Work out the finished part from the listing and answer in its coordinate system (mm). Give positions to 0.01 mm unless a question says otherwise; leave off trailing zeros. Order: outer loops, then holes, each group sorted by start corner. A loop starts at its lowest first (then second) coordinate and runs counter-clockwise, first axis right, second up. Notation, with made-up numbers: (80, 50.25) -> (90, 50.25) arc R24 cw to (90, 87.25) -> close; hole circle Ø6 at (-23, 40). An arc over 180 degrees is marked (long way). Answer as CSV lines item,"result". Start each with the question number.
1. A cutting plane is placed at A-A (y = 316). Give the vertices of the cut face in (x, z), then the cut area to 3 significant figures.
2. A flat-ended cylindrical pin translates along its axis: pin 1 (6 mm diameter, centred on x = 29, y = 284.5, fed in from +Z). Find the tip coordinate at first contact, or state that the pin passes through.
3. A cutting plane is placed at B-B (x = -35). Give the vertices of the cut face in (y, z) (3 decimals).
4. Find the intervals of material crossed by L1, parallel to Z at x = -33.5, y = 298; L2, parallel to Z at x = -36, y = 370; L3, parallel to X at y = 58.5, z = -35 (3 decimals), in increasing order.
5. A cutting plane is placed at C-C (z = 34.5). Give the vertices of the cut face in (x, y).
from build123d import *

# Parameters (mm, degrees)
BOSS_EXTRUDE1_DEPTH = 420


with BuildPart() as part:
    # Sketch1 → Boss-Extrude1 (new body)
    with BuildSketch(Plane.XZ):
        with BuildLine():
            Line((40, -26.666666667), (40, 26.666666667))
            ThreePointArc((40, 26.666666667), (36.094757082, 36.094757082), (26.666666667, 40))
            Line((26.666666667, 40), (-26.666666667, 40))
            ThreePointArc((-26.666666667, 40), (-36.094757082, 36.094757082), (-40, 26.666666667))
            Line((-40, 26.666666667), (-40, -26.666666667))
            ThreePointArc((-40, -26.666666667), (-36.094757082, -36.094757082), (-26.666666667, -40))
            Line((-26.666666667, -40), (26.666666667, -40))
            ThreePointArc((26.666666667, -40), (36.094757082, -36.094757082), (40, -26.666666667))
        make_face()
    extrude(amount=-BOSS_EXTRUDE1_DEPTH)


solid = part.part
Answer sheet:
1,outline,"(-40, -26.67) arc R13.33 ccw to (-26.67, -40) -> (26.67, -40) arc R13.33 ccw to (40, -26.67) -> (40, 26.67) arc R13.33 ccw to (26.67, 40) -> (-26.67, 40) arc R13.33 ccw to (-40, 26.67) -> close"
1,area,"6,250 mm^2"
2,pin 1,"stops at z = 40"
3,outline,"(0, -37.075) -> (420, -37.075) -> (420, 37.075) -> (0, 37.075) -> close"
4,L1,"z = -38.12 to 38.12"
4,L2,"z = -36.19 to 36.19"
4,L3,"x = -37.075 to 37.075"
5,outline,"(-37.46, 0) -> (37.46, 0) -> (37.46, 420) -> (-37.46, 420) -> close"
